from build123d import *

# Parameters (mm, degrees)
SKETCH_1_W          = 30
SKETCH_1_H          = 40
EXTRUDE_1_DEPTH     = 30
SKETCH_4_W          = 20
SKETCH_4_H          = 35
CUT_EXTRUDE_1_DEPTH = 40
CUT_EXTRUDE_2_DEPTH = 40
SKETCH_6_R          = 2.5
CUT_EXTRUDE_3_DEPTH = 40
SKETCH_7_R          = 4
CUT_EXTRUDE_4_DEPTH = 40


with BuildPart() as part:
    # 草图1 → 凸台-拉伸1 (new body)
    with BuildSketch(Plane.XY):
        with Locations((15, 20)):
            Rectangle(SKETCH_1_W, SKETCH_1_H)
    extrude(amount=EXTRUDE_1_DEPTH)

    # 草图4 → 切除-拉伸1 (cut)
    with BuildSketch(Plane(origin=(30, 0, 0), x_dir=(0, 0, -1), z_dir=(1, 0, 0))):
        with Locations((-15, 22.5)):
            Rectangle(SKETCH_4_W, SKETCH_4_H)
    extrude(amount=-CUT_EXTRUDE_1_DEPTH, mode=Mode.SUBTRACT)

    # 草图5 → 切除-拉伸2 (cut)
    with BuildSketch(Plane(origin=(0, 0, 0), x_dir=(-1, 0, 0), z_dir=(0, 0, -1))):
        with BuildLine():
            Line((-30, 20), (-30, 40))
            Line((-30, 40), (0, 40))
            Line((0, 40), (0, 20))
            ThreePointArc((0, 20), (-15, 35), (-30, 20))
        make_face()
    extrude(amount=-CUT_EXTRUDE_2_DEPTH, mode=Mode.SUBTRACT)

    # 草图6 → 切除-拉伸3 (cut)
    with BuildSketch(Plane(origin=(0, 0, 0), x_dir=(-1, 0, 0), z_dir=(0, 0, -1))):
        with Locations((-15, 28)):
            Circle(SKETCH_6_R)
    extrude(amount=-CUT_EXTRUDE_3_DEPTH, mode=Mode.SUBTRACT)

    # 草图7 → 切除-拉伸4 (cut)
    with BuildSketch(Plane.XZ):
        with Locations(Location((15, 15, 0), (0, 0, 270))):
            Circle(SKETCH_7_R)
    extrude(amount=-CUT_EXTRUDE_4_DEPTH, mode=Mode.SUBTRACT)


solid = part.part
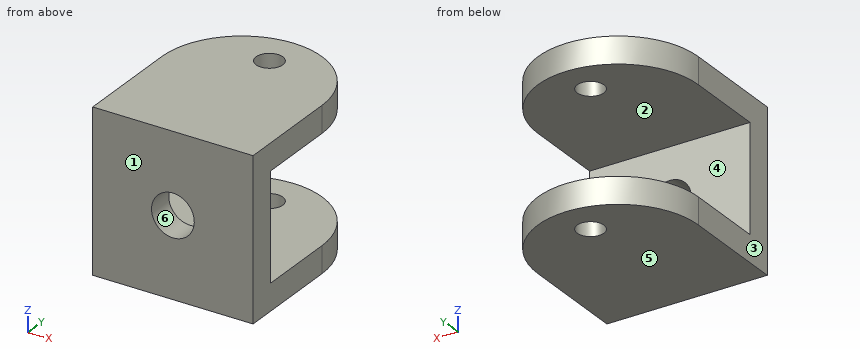
Can you work these out from the model? Positions are in its coordinate system, mm. Face numbers are marked on the shaded views. A direction names the side the tool comes from. Give positions to 0.01 mm unless a question says otherwise; leave off trailing zeros. Order: outer loops, then holes, each group sorted by start corner. A loop starts at its lowest first (then second) coordinate and runs counter-clockwise, first axis right, second up. Notation, with made-up numbers: M -4.75,-13.75 L 51.25,-13.75 A23 cw 51.25,24.25 Z; hole C 52.5,73.25 d8. An arc over 180 degrees is marked long. Use one line per item in the form item = value. Start each with the question number.
Item 1: We'd pull the mould along Z, two halves only. Please class the marked faces 3, 4, 5 and 6: +Z half, -Z half, draft (parallel to the pull), parting line (faces both ways), or undercut.
Item 2: If we section it at B-B (y = 15.5): Write out the boundary of the cut face in (x, z).
Item 3: For the marked faces 1 and 2, which set-ups out of +Z, -Z, +X, -X, +Y, -Y let a thin tool reach every point of the face, with its end or its side?
Item 4: If I drill on line 1 along Z through (x, y) = (12.25, 20); line 2 along Y through (x, z) = (15, 2.85); line 3 along X through (y, z) = (3.5, 15), over which ranges is the centre line in solid material (lowest first)?
Item 5: If we section it at C-C (x = 15): Write out the boundary of the cut face in (y, z).
Item 6: If we section it at D-D (y = 28): Write out the boundary of the cut face in (x, z), then the cut area to 3 significant figures.
Item 7: If we section it at A-A (z = 15): Write out the boundary of the cut face in (x, y), then the cut area to 3 significant figures.
Outcome:
q1.face_3 = draft
q1.face_4 = undercut
q1.face_5 = -Z half
q1.face_6 = undercut
q2.outline = M 0,0 L 30,0 L 30,5 L 0,5 Z; M 0,25 L 30,25 L 30,30 L 0,30 Z
q3.face_1 = +Z, -Z, +X, -X, -Y
q3.face_2 = +X, -X, +Y
q4.line_1 = 0 to 5, 25 to 30
q4.line_2 = 0 to 25.5, 30.5 to 35
q4.line_3 = 0 to 11, 19 to 30
q5.outline = M 0,0 L 25.5,0 L 25.5,5 L 5,5 L 5,11 L 0,11 Z; M 0,19 L 5,19 L 5,25 L 25.5,25 L 25.5,30 L 0,30 Z; M 30.5,0 L 35,0 L 35,5 L 30.5,5 Z; M 30.5,25 L 35,25 L 35,30 L 30.5,30 Z
q6.outline = M 2.31,0 L 12.5,0 L 12.5,5 L 2.31,5 Z; M 2.31,25 L 12.5,25 L 12.5,30 L 2.31,30 Z; M 17.5,0 L 27.69,0 L 27.69,5 L 17.5,5 Z; M 17.5,25 L 27.69,25 L 27.69,30 L 17.5,30 Z
q6.area = 204 mm2
q7.outline = M 0,0 L 11,0 L 11,5 L 0,5 Z; M 19,0 L 30,0 L 30,5 L 19,5 Z
q7.area = 110 mm2
